Could you check a few things on this model? Use its own coordinates, in mm. Give positions to 0.01 mm unless a question says otherwise; leave off trailing zeros. Loops run counter-clockwise (first coordinate to the right, second up) from the corner with the lowest first, then second, coordinate; pieces in that order, holes last. Notation, with made-up numbers: M 26,26 L 34,26 A35 cw 34,59 Z; hole C -8,32.5 d3. An arc over 180 degrees is marked long. Use a Markdown table: item, result. Add a question column.
1) Suppose I cut it at B-B on x = 119.5. List the corners of the cut face in (y, z) for me, and give its area (3 significant figures).
2) Suppose I cut it at C-C on y = 220. List the corners of the cut face in (x, z) for me, and give its area (3 significant figures).
3) Will these pins go through, and if not, where does the flat tip stop? pin 1 Ø8 at (y, z) = (48.5, 13) entering from -X; pin 2 Ø8 at (x, z) = (47, 6) entering from -Y; pin 3 Ø7.5 at (x, z) = (38, 6) entering from +Y.
4) Suppose I cut it at A-A on z = 6. Count the separate pieces of the cut face and the enclosed holes in it, and give its area (3 significant figures).
5) If I drill on line 1 along Y through (x, z) = (0, 4.5); line 2 along Y through (x, z) = (14, 0.75); line 3 along X through (y, z) = (104, 13), over which ranges is the centre line in solid material (lowest first)? Write a range as [from, to].
```python
from build123d import *

# Parameters (mm, degrees)
SKETCH_1_R      = 2
SKETCH_1_R_2    = 16
SKETCH_1_R_3    = 3.91899873
SKETCH_1_R_4    = 3
EXTRUDE_3_DEPTH = 15


with BuildPart() as part:
    # 草图1 → 凸台-拉伸3 (new body)
    with BuildSketch(Plane.XY):
        with BuildLine():
            Line((-14, 116), (-6, 0))
            ThreePointArc((-6, 0), (0, -6), (6, 0))
            add(Edge.make_bspline(
                [(6, 0), (1.588652615, 45.680929706), (5.604102499, 67.643200211), (28.004797731, 100.13093391)],
                knots=[0, 0, 0, 0, 0.788155359, 0.788155359, 0.788155359, 0.788155359], degree=3))
            ThreePointArc((28.004797731, 100.13093391), (50.113637924, 116.900750568), (77, 123.767416406))
            ThreePointArc((77, 123.767416406), (157.787149523, 158.485384951), (196.379869136, 237.494896157))
            ThreePointArc((196.379869136, 237.494896157), (200.439238403, 240.311917913), (202, 245))
            Line((202, 245), (202, 250))
            ThreePointArc((202, 250), (194.5, 257.5), (187, 250))
            ThreePointArc((187, 250), (154.781745931, 172.218254069), (77, 140))
            Line((77, 140), (10, 140))
            ThreePointArc((10, 140), (-6.970562748, 132.970562748), (-14, 116))
        make_face()
        Circle(SKETCH_1_R, mode=Mode.SUBTRACT)
        with Locations((10, 116)):
            Circle(SKETCH_1_R_2, mode=Mode.SUBTRACT)
        with Locations((194.5, 250)):
            Circle(SKETCH_1_R_3, mode=Mode.SUBTRACT)
        with Locations((0, 22)):
            Circle(SKETCH_1_R_4, mode=Mode.SUBTRACT)
    extrude(amount=EXTRUDE_3_DEPTH)


solid = part.part
```
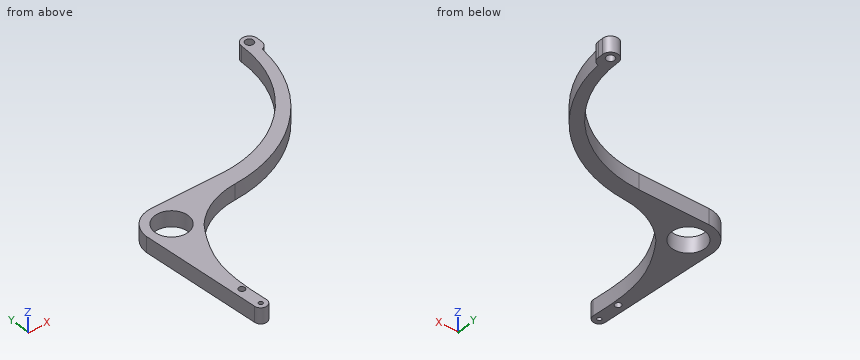
Answer block:
| question | item | result |
|---|---|---|
| 1 | outline | M 133.45,0 L 148.54,0 L 148.54,15 L 133.45,15 Z |
| 1 | area | 226 mm^2 |
| 2 | outline | M 182.83,0 L 193.39,0 L 193.39,15 L 182.83,15 Z |
| 2 | area | 158 mm^2 |
| 3 | pin 1 | stops at x = -9.62 |
| 3 | pin 2 | stops at y = 112.94 |
| 3 | pin 3 | stops at y = 140 |
| 4 | separate pieces | 1 |
| 4 | enclosed holes | 4 |
| 4 | area | 6,190 mm^2 |
| 5 | line 1 | y = [-6, -2], [2, 19], [25, 103.51], [128.49, 137.82] |
| 5 | line 2 | y = [76.14, 100.51], [131.49, 140] |
| 5 | line 3 | x = [-13.17, -0.58], [20.58, 31.69] |
